For this review, take the finished solid that the model builds, in its own axes (mm). Face numbers are marked on the shaded views. Coordinates: 2 decimals unless noted, no trailing zeros. Write each loop counter-clockwise with the first axis right and the second up, starting at its lowest first coordinate (ties: lowest second). Pieces come first, ordered by that corner, then holes.
1) To check wall thickness, follow line 1 along X through (y, z) = (23, 10.5); line 2 along Y through (x, z) = (13.75, 13.75); line 3 along Y through (x, z) = (0.5, 20.75). State the ranges of each line that lie inside material, in increasing order.
2) We need section B-B on x = 13. Write out the cut boundary in (y, z), then the cut area to 3 significant figures.
3) Mouldability with a two-part tool opening along Y and no side actions: class the marked faces 1 and 2 as pulls with the +Y half, pulls with the -Y half, needs draft (parallel to the pull), parting line crosses it, or undercut.
4) Insertion check: P1, Ø6, axis at x = 3.5, z = 18, coming from the +Y side; P2, Ø1, axis at x = 0.5, z = 6, coming from the -Y side; P3, Ø8, axis at y = 58, z = 4, coming from the +X side; P4, Ø2, axis at x = 6, y = 41, coming from the +Z side. Each pin has a flat end and moves straight along its axis. Give the tip position at first contact, or say it passes through.
5) We need section A-A on z = 6. Write out the cut boundary in (x, y).
6) We need section D-D on x = 3.25. Write out the cut boundary in (y, z), then the cut area to 3 significant figures.
7) We need section C-C on y = 42.5. Write out the cut boundary in (x, z).
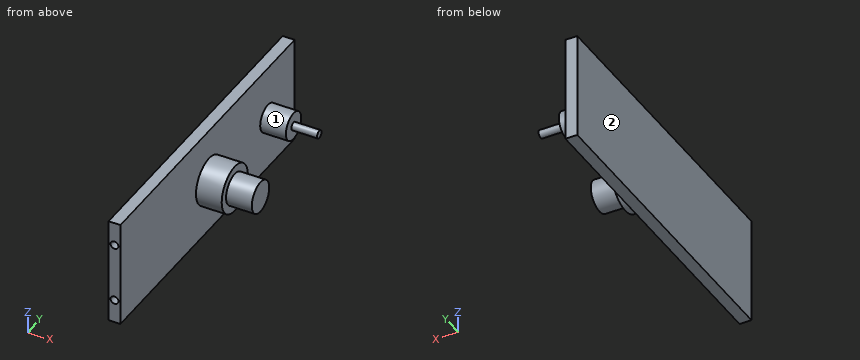
from build123d import *

# Parameters (mm, degrees)
SKETCH_1_W          = 3
SKETCH_1_H          = 80
EXTRUDE_1_DEPTH     = 27
SKETCH_2_R          = 3.5
SKETCH_2_R_2        = 6
EXTRUDE_2_DEPTH     = 6.5
SKETCH_3_R          = 1
SKETCH_3_R_2        = 4
EXTRUDE_3_DEPTH     = 6.5
SKETCH_4_R          = 1
CUT_EXTRUDE_1_DEPTH = 15


with BuildPart() as part:
    # 草图1 → 凸台-拉伸1 (new body)
    with BuildSketch(Plane.XY):
        with Locations((0.517241379, 39.071316614)):
            Rectangle(SKETCH_1_W, SKETCH_1_H)
    extrude(amount=EXTRUDE_1_DEPTH)

    # 草图2 → 凸台-拉伸2 (add)
    with BuildSketch(Plane(origin=(2.017241379, 0, 0), x_dir=(0, 0, -1), z_dir=(1, 0, 0))):
        with Locations(Location((-13.5, 66.771316614, 0), (0, 0, 270))):
            Circle(SKETCH_2_R)
        with Locations(Location((-13.5, 39.771316614, 0), (0, 0, 270))):
            Circle(SKETCH_2_R_2)
    extrude(amount=EXTRUDE_2_DEPTH)

    # 草图3 → 凸台-拉伸3 (add)
    with BuildSketch(Plane(origin=(8.517241379, 0, 0), x_dir=(0, 0, -1), z_dir=(1, 0, 0))):
        with Locations(Location((-13.5, 66.771316614, 0), (0, 0, 270))):
            Circle(SKETCH_3_R)
        with Locations(Location((-13.5, 39.771316614, 0), (0, 0, 270))):
            Circle(SKETCH_3_R_2)
    extrude(amount=EXTRUDE_3_DEPTH)

    # 草图4 → 切除-拉伸1 (cut)
    with BuildSketch(Plane(origin=(-1096.213929055, -10.928683386, 855.0606199), x_dir=(0.12186934340512692, -2.2319547324357124e-14, -0.9925461516413246), z_dir=(0, -1, 0))):
        with Locations((963.085867609, 999.8129825)):
            Circle(SKETCH_4_R)
        with Locations((977.974059883, 997.984942349)):
            Circle(SKETCH_4_R)
        with Locations(Location((961.501566145, 986.909882529, 0), (0, 0, 83))):
            Circle(SKETCH_4_R)
        with Locations(Location((976.389758419, 985.081842378, 0), (0, 0, 83))):
            Circle(SKETCH_4_R)
    extrude(amount=-CUT_EXTRUDE_1_DEPTH, mode=Mode.SUBTRACT)


solid = part.part
Result:
1. line 1: x = -0.98 to 2.02
1. line 2: y = 35.78 to 43.76, 65.8 to 67.74
1. line 3: y = 4.07 to 79.07
2. outline: circle Ø8 at (39.77, 13.5); circle Ø2 at (66.77, 13.5)
2. area: 53.4 mm2
3. face 1: undercut
3. face 2: needs draft
4. P1: stops at y = 79.07
4. P2: stops at y = 4.07
4. P3: stops at x = 2.02
4. P4: stops at z = 19.5
5. outline: (-0.98, -0.93) - (-0.48, -0.93) - (-0.48, 4.07) - (1.52, 4.07) - (1.52, -0.93) - (2.02, -0.93) - (2.02, 79.07) - (-0.98, 79.07) - close
6. outline: circle Ø12 at (39.77, 13.5); circle Ø7 at (66.77, 13.5)
6. area: 152 mm2
7. outline: (-0.98, 0) - (2.02, 0) - (2.02, 8.16) - (8.52, 8.16) - (8.52, 10.58) - (15.02, 10.58) - (15.02, 16.42) - (8.52, 16.42) - (8.52, 18.84) - (2.02, 18.84) - (2.02, 27) - (-0.98, 27) - close
